from build123d import *

# Parameters (mm, degrees)
BOSS_EXTRUDE1_DEPTH = 2.7


with BuildPart() as part:
    # Sketch1 → Boss-Extrude1 (new body)
    with BuildSketch(Plane.XY):
        with BuildLine():
            Line((-14.696938457, 24.985281374), (-16.887495374, 26.25))
            ThreePointArc((-16.887495374, 26.25), (-18.199948236, 23.500848821), (-19.068213964, 20.580835235))
            Line((-19.068213964, 20.580835235), (-15.186057607, 18.339471217))
            ThreePointArc((-15.186057607, 18.339471217), (-13.000189211, 18.186313351), (-11.533289054, 19.814097705))
            ThreePointArc((-11.533289054, 19.814097705), (9.5856448, 23.719100621), (0, 4.5))
            ThreePointArc((0, 4.5), (-4.5, 0), (0, -4.5))
            ThreePointArc((0, -4.5), (9.5856448, -23.719100621), (-11.533289054, -19.814097705))
            ThreePointArc((-11.533289054, -19.814097705), (-13.000189211, -18.186313351), (-15.186057607, -18.339471217))
            Line((-15.186057607, -18.339471217), (-19.068213964, -20.580835235))
            ThreePointArc((-19.068213964, -20.580835235), (-18.199948236, -23.500848821), (-16.887495374, -26.25))
            Line((-16.887495374, -26.25), (-14.696938457, -24.985281374))
            ThreePointArc((-14.696938457, -24.985281374), (-13.966653368, -24.87818357), (-13.36182443, -25.301229909))
            ThreePointArc((-13.36182443, -25.301229909), (14.085802756, -24.088818138), (0, -0.5))
            ThreePointArc((0, -0.5), (-0.5, 0), (0, 0.5))
            ThreePointArc((0, 0.5), (14.085802756, 24.088818138), (-13.36182443, 25.301229909))
            ThreePointArc((-13.36182443, 25.301229909), (-13.966653368, 24.87818357), (-14.696938457, 24.985281374))
        make_face()
    extrude(amount=BOSS_EXTRUDE1_DEPTH)


solid = part.part
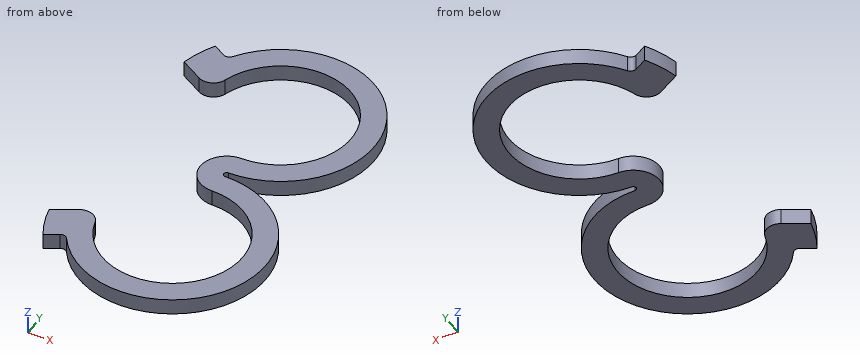
Design review of the part built by this model. Coordinates are the model's own, in mm. Coordinates: 2 decimals unless noted, no trailing zeros. Order: outer loops, then holes, each group sorted by start corner. A loop starts at its lowest first (then second) coordinate and runs counter-clockwise, first axis right, second up. Notation, with made-up numbers: (56, 65.25) -> (115, 65.25) arc R21 ccw to (115, 69.25) -> close; hole circle Ø1 at (56, -27). An arc over 180 degrees is marked (long way). Use one line per item in the form item = value. Start each with the question number.
(1) Add section D-D on y = 9.5. State the section outline as (x, z) points.
(2) For probe 1 along Y at (x, z) = (-1.5, 2.65); probe 2 along X at (y, z) = (-16.5, 1.1); probe 3 along X at (y, z) = (-22.5, 0.6), list the stretches that pass through material, from the lowest coordinate up.
(3) Add section C-C on y = 16.5. State the section outline as (x, z) points, plus the area to 3 significant figures.
(4) Add section A-A on x = -2. State the section outline as (y, z) points.
(5) Insertion check: pin 1 (8 mm diameter, centred on x = -8.5, y = 16.5, fed in from -Z). The pin has a flat end and moves straight along its axis. Give the tip position at first contact, or say it passes through.
(6) Add section B-B on z = 1.6. State the section outline as (x, y) points, plus the area to 3 significant figures.
Answer block:
q1.outline = (9.75, 0) -> (14.39, 0) -> (14.39, 2.7) -> (9.75, 2.7) -> close
q2.probe_1 = -32.43 to -28.41, -4.24 to 4.24, 28.41 to 32.43
q2.probe_2 = 12 to 16
q2.probe_3 = -18.55 to -10.39, 10.39 to 14.83
q3.outline = (12, 0) -> (16, 0) -> (16, 2.7) -> (12, 2.7) -> close
q3.area = 10.8 mm²
q4.outline = (-32.37, 0) -> (-28.33, 0) -> (-28.33, 2.7) -> (-32.37, 2.7) -> close; (-4.03, 0) -> (4.03, 0) -> (4.03, 2.7) -> (-4.03, 2.7) -> close; (28.33, 0) -> (32.37, 0) -> (32.37, 2.7) -> (28.33, 2.7) -> close
q5.pin_1 = through
q6.outline = (-19.07, -20.58) arc R19.5 ccw to (-16.89, -26.25) -> (-14.7, -24.99) arc R1 cw to (-13.36, -25.3) arc R16 ccw (long way) to (0, -0.5) arc R0.5 cw to (0, 0.5) arc R16 ccw (long way) to (-13.36, 25.3) arc R1 cw to (-14.7, 24.99) -> (-16.89, 26.25) arc R19.5 ccw to (-19.07, 20.58) -> (-15.19, 18.34) arc R2.5 ccw to (-11.53, 19.81) arc R12 cw (long way) to (0, 4.5) arc R4.5 ccw to (0, -4.5) arc R12 cw (long way) to (-11.53, -19.81) arc R2.5 ccw to (-15.19, -18.34) -> close
q6.area = 588 mm²
